Check sheet for the modelled part. Datum: model origin and axes. Units: mm. A direction names the side the tool comes from. Coordinates: 2 decimals unless noted, no trailing zeros. Loops run counter-clockwise (first coordinate to the right, second up) from the corner with the lowest first, then second, coordinate; pieces in that order, holes last. Notation, with made-up numbers: M 19.5,63.5 L 44.5,63.5 A20 cw 44.5,82.5 Z; hole C 71.25,29.5 d5. An arc over 180 degrees is marked long. Return JSON: item names as keys, results as strings.
from build123d import *

# Parameters (mm, degrees)
SKETCH_1_W               = 1080
SKETCH_1_H               = 200
EXTRUDE_1_DEPTH          = 150
SKETCH_2_R               = 135
SKETCH_2_R_2             = 150
CUT_EXTRUDE_1_DEPTH      = 130
CUT_EXTRUDE_2_DEPTH      = 570.2978131
CUT_EXTRUDE_2_DEPTH_BACK = 570.2978131
SKETCH_2_3_R             = 125
SKETCH_2_3_R_2           = 135


with BuildPart() as part:
    # 草图1 → 凸台-拉伸1 (new body)
    with BuildSketch(Plane.XY):
        Rectangle(SKETCH_1_W, SKETCH_1_H)
    extrude(amount=EXTRUDE_1_DEPTH)

    # 草图2 → 切除-拉伸1 (cut)
    with BuildSketch(Plane.XY.offset(150)):
        with Locations((-280, -100)):
            Circle(SKETCH_2_R)
        with Locations((220, -100)):
            Circle(SKETCH_2_R_2)
    extrude(amount=-CUT_EXTRUDE_1_DEPTH, mode=Mode.SUBTRACT)

    # 草图2<3> → 切除-拉伸2 (cut, two sides: drawn at the far end of the back side and taken through both)
    with BuildSketch(Plane.XY.offset(150).offset(-CUT_EXTRUDE_2_DEPTH_BACK)):
        with Locations((-280, -100)):
            Circle(SKETCH_2_3_R)
        with Locations((220, -100)):
            Circle(SKETCH_2_3_R_2)
    extrude(amount=CUT_EXTRUDE_2_DEPTH + CUT_EXTRUDE_2_DEPTH_BACK, mode=Mode.SUBTRACT)


solid = part.part
1) Section check A-A on y = -23. Record the cut outline in (x, z), then the cut area to 3 significant figures.
Answers:
{"outline": "M -540,0 L -378.47,0 L -378.47,20 L -390.89,20 L -390.89,150 L -540,150 Z; M -181.53,0 L 109.11,0 L 109.11,20 L 91.27,20 L 91.27,150 L -169.11,150 L -169.11,20 L -181.53,20 Z; M 330.89,0 L 540,0 L 540,150 L 348.73,150 L 348.73,20 L 330.89,20 Z", "area": "91,300 mm²"}
2) Section check B-B on x = 220. Record the cut outline in (y, z), then the cut area to 3 significant figures.
Answers:
{"outline": "M 35,0 L 100,0 L 100,150 L 50,150 L 50,20 L 35,20 Z", "area": "7,800 mm²"}
3) Section check C-C on z = 71. Record the cut outline in (x, y), then the cut area to 3 significant figures.
Answers:
{"outline": "M -540,-100 L -415,-100 A135 cw -145,-100 L 70,-100 A150 cw 370,-100 L 540,-100 L 540,100 L -540,100 Z", "area": "152,000 mm²"}
4) Set-up check for faces 1 (the face through (223.298, 49.964, 85.91)), 2 (the face through (540, -1, 74)): record each of +Z, -Z, +X, -X, +Y, -Y from which the full face is reachable in a straight line by a thin tool's end or side.
Answers:
{"face 1": "+Z, -Y", "face 2": "+Z, -Z, +X, +Y, -Y"}
5) Section check D-D on y = -80.5. Record the cut outline in (x, z).
Answers:
{"outline": "M -540,0 L -403.47,0 L -403.47,20 L -413.58,20 L -413.58,150 L -540,150 Z; M -156.53,0 L 86.42,0 L 86.42,20 L 71.27,20 L 71.27,150 L -146.42,150 L -146.42,20 L -156.53,20 Z; M 353.58,0 L 540,0 L 540,150 L 368.73,150 L 368.73,20 L 353.58,20 Z"}
6) Scan lines: line 1 along X through (y, z) = (-20.5, 88); line 2 along X through (y, z) = (6, 47); line 3 along Y through (x, z) = (-283.5, 127). Record each from-to range of solid material in increasing order. Write a range as [from, to].
Answers:
{"line 1": "[-540, -389.11], [-170.89, 92.8], [347.2, 540]", "line 2": "[-540, -363.6], [-196.4, 113.87], [326.13, 540]", "line 3": "[34.95, 100]"}
7) Draft check along X on faces 3 (the face through (222.969, 34.967, 9.86)), 4 (the face through (-8, 24, 0)), 5 (the face through (-540, -1, 74)). Enter one of: +X half, -X half, draft (parallel to the pull), parting line (faces both ways), or undercut.
Answers:
{"face 3": "undercut", "face 4": "draft", "face 5": "-X half"}
8) Go/stop test with flat-tipped pins: pin 1 Ø10 at (x, z) = (-218, 32) entering from -Y; pin 2 Ø2 at (x, y) = (218.5, 45.5) entering from +Z; pin 3 Ø1 at (x, z) = (-208.5, 86) entering from -Y. Record where each tip stops, or that it passes through.
Answers:
{"pin 1": "y = 17.2", "pin 2": "z = 20", "pin 3": "y = 14.2"}
